Answer from the drawing. Dimensions are ordinates in mm from the lowest x, y and z of the part. A direction names the side the tool comes from. Give positions to 0.01 mm unless a question says otherwise; leave off trailing zeros. Loops run counter-clockwise (first coordinate to the right, second up) from the corner with the lowest first, then second, coordinate; pieces in that order, holes last. Notation, with made-up numbers: (55, 75) -> (59, 75) arc R37 ccw to (59, 114) -> close; hole circle Ø2 at (20.5, -2). An arc over 180 degrees is marked (long way). Return JSON: item names as keys, results as strings. Group by question number.
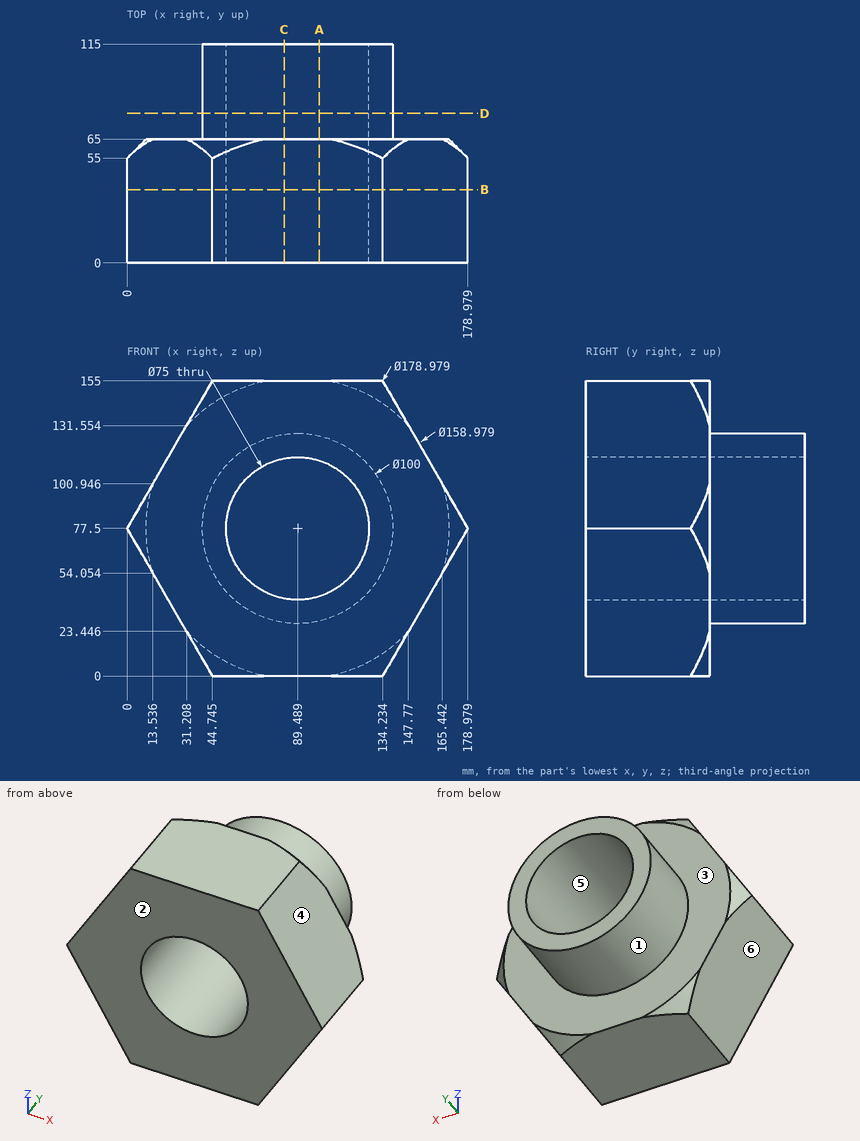
1. Section D-D on y = 78.5 is taken. Determine the outline of the cut face in (x, z), then the cut area to 3 significant figures.
2. Section C-C on x = 82.5 is taken. Determine the outline of the cut face in (y, z), then the cut area to 3 significant figures.
3. Which of the six approach directions +Z, -Z, +X, -X, +Y, -Y give full straight-line access (tool end or side, diameter ignored) to the marked faces 1 and 2?
4. Section A-A on x = 101 is taken. Determine the outline of the cut face in (y, z).
5. Flat-ended cylindrical pins translate along their axes: pin 1 Ø3 at (y, z) = (85, 98.5) entering from -X; pin 2 Ø12 at (y, z) = (20, 129.5) entering from +X; pin 3 Ø1 at (x, y) = (158.5, 62.5) entering from +Z (1 decimal). Find the tip coordinate at first contact, or state that the pin passes through.
6. Section B-B on y = 38.5 is taken. Determine the outline of the cut face in (x, z) (1 decimal).
7. Determine the mould class of the marked faces 3, 4, 5 and 6 for opening direction Z: pulls with the +Z half, pulls with the -Z half, needs draft (parallel to the pull), parting line crosses it, or undercut.
8. Straight lines are drawn through the part: line 1 (Z direction, x = 89, y = 104); line 2 (X direction, y = 36.5, z = 77.5); line 3 (Y direction, x = 148, z = 108.5). For each, find the intervals that lie inside material, in ascending order. Write a range as from..to.
Completed:
{
 "1": {"outline": "circle Ø100 at (89.49, 77.5); hole circle Ø75 at (89.49, 77.5)", "area": "3,440 mm²"},
 "2": {"outline": "(0, 0) -> (65, 0) -> (65, 27.99) -> (115, 27.99) -> (115, 40.66) -> (0, 40.66) -> close; (0, 114.34) -> (115, 114.34) -> (115, 127.01) -> (65, 127.01) -> (65, 155) -> (0, 155) -> close", "area": "6,550 mm²"},
 "3": {"face 1": "+Y", "face 2": "+Z, -Z, +X, -X, -Y"},
 "4": {"outline": "(0, 0) -> (65, 0) -> (65, 28.84) -> (115, 28.84) -> (115, 41.81) -> (0, 41.81) -> close; (0, 113.19) -> (115, 113.19) -> (115, 126.16) -> (65, 126.16) -> (65, 155) -> (0, 155) -> close"},
 "5": {"pin 1": "stops at x = 43.45", "pin 2": "stops at x = 152.42", "pin 3": "stops at z = 113.8"},
 "6": {"outline": "(0, 77.5) -> (44.7, 0) -> (134.2, 0) -> (179, 77.5) -> (134.2, 155) -> (44.7, 155) -> close; hole circle Ø75 at (89.5, 77.5)"},
 "7": {"face 3": "needs draft", "face 4": "pulls with the +Z half", "face 5": "undercut", "face 6": "pulls with the -Z half"},
 "8": {"line 1": "z = 27.5..40, 115..127.5", "line 2": "x = 0..51.99, 126.99..178.98", "line 3": "y = 0..65"}
}
